Part print with two shaded views. Sizes in mm from the minimum x, y, z corner. A direction names the side the tool comes from. Give positions to 0.01 mm unless a question says otherwise; leave off trailing zeros. Write each loop counter-clockwise with the first axis right and the second up, starting at its lowest first coordinate (ties: lowest second). Pieces come first, ordered by that corner, then holes. Notation, with made-up numbers: (-9, 0.25) - (-4, 0.25) arc R23 ccw to (-4, 12.25) - close; hole circle Ø2 at (-26, -11.5). An arc over 180 degrees is marked (long way). Answer as a JSON object with one key per item and string values.
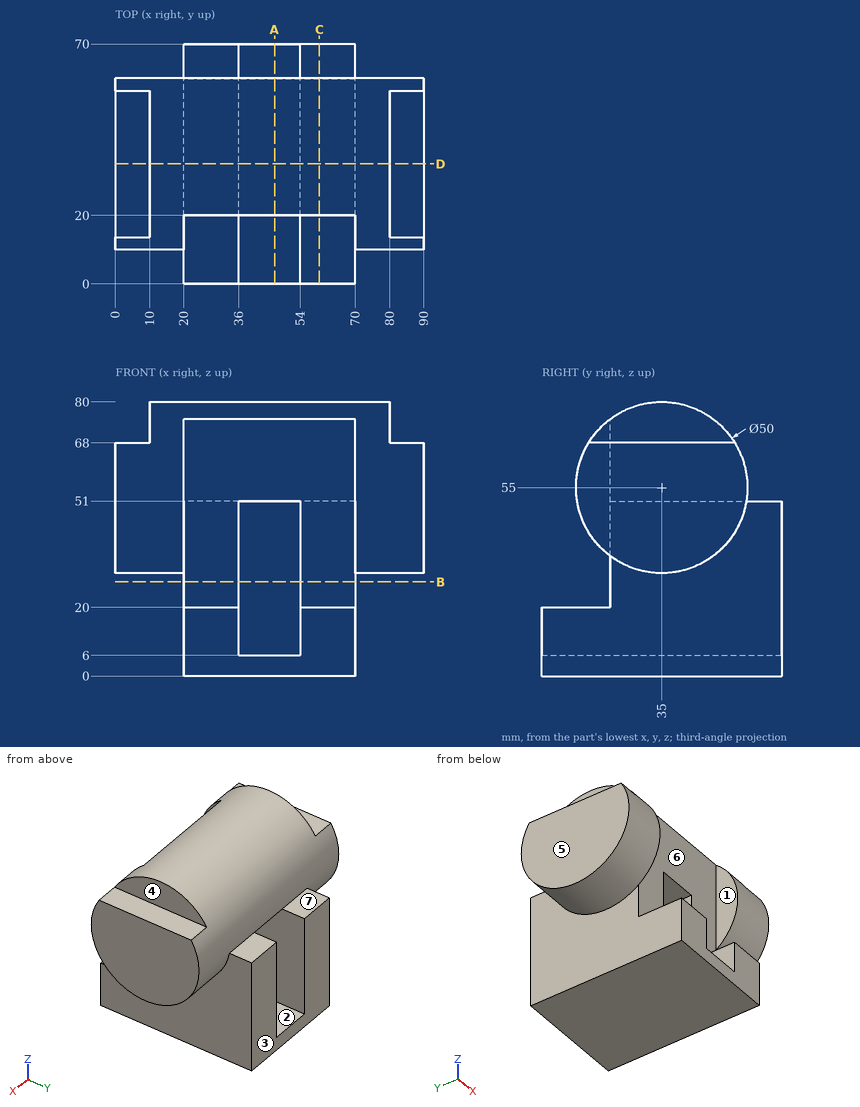
(1) Probe L1, parallel to X at y = 18, z = 37; L2, parallel to X at y = 44, z = 19; L3, parallel to X at y = 36, z = 75. List the from-to ranges inside material, lowest first. Write a range as [from, to].
Answer key:
{"L1": "x = [0, 20], [70, 90]", "L2": "x = [20, 36], [54, 70]", "L3": "x = [10, 80]"}
(2) 3-axis set-ups, long thin cutter, end or side, ignore diameter. For the marked faces 1, 2, 3 and 4: which of +Z, -Z, +X, -X, +Y, -Y reach the whole face in a straight line?
Answer key:
{"face 1": "+Z, -Y", "face 2": "+Y, -Y", "face 3": "+Z, -Z, +X, -X, +Y", "face 4": "+Z, +X, +Y, -Y"}
(3) Saw through at B-B, the plane z = 27.5. Give the cut face in (x, y), and give its area (3 significant figures).
Answer key:
{"outline": "(20, 20) - (36, 20) - (36, 70) - (20, 70) - close; (54, 20) - (70, 20) - (70, 70) - (54, 70) - close", "area": "1,600 mm²"}
(4) Pull direction X, two halves, no side cores. Call the marked faces 5, 6 and 7: pulls with the +X half, pulls with the -X half, needs draft (parallel to the pull), parting line crosses it, or undercut.
Answer key:
{"face 5": "pulls with the -X half", "face 6": "undercut", "face 7": "needs draft"}
(5) Saw through at D-D, the plane y = 35. Give the cut face in (x, z).
Answer key:
{"outline": "(0, 30) - (20, 30) - (20, 0) - (70, 0) - (70, 30) - (90, 30) - (90, 68) - (80, 68) - (80, 80) - (10, 80) - (10, 68) - (0, 68) - close; hole (36, 6) - (54, 6) - (54, 51) - (36, 51) - close"}
(6) Saw through at A-A, the plane x = 46.5. Give the cut face in (y, z), and give its area (3 significant figures).
Answer key:
{"outline": "(0, 0) - (70, 0) - (70, 6) - (0, 6) - close; (20, 51) - (59.68, 51) arc R25 ccw to (20, 75) - close", "area": "1,420 mm²"}
(7) Saw through at C-C, the plane x = 59.5. Give the cut face in (y, z).
Answer key:
{"outline": "(0, 0) - (70, 0) - (70, 51) - (59.68, 51) arc R25 ccw to (20, 75) - (20, 20) - (0, 20) - close"}
(8) Flat gauge pins, fed straight in: P1, Ø17.5, axis at x = 27, y = 10.5, coming from the +Z side; P2, Ø3.5, axis at y = 40, z = 72.5, coming from the +X side; P3, Ø3, axis at x = 66, y = 65, coming from the +Z side. Where does each tip first touch, or does it go through?
Answer key:
{"P1": "stops at z = 70.95", "P2": "stops at x = 80", "P3": "stops at z = 51"}
